```python
from build123d import *

# Parameters (mm, degrees)
SKETCH_1_R             = 12.5
EXTRUDE_1_DEPTH        = 298
SKETCH_2_R             = 10
EXTRUDE_2_DEPTH        = 56
EXTRUDE_START          = 56
SKETCH_3_R             = 10
EXTRUDE_3_DEPTH        = 56
SKETCH_4_R             = 7.5
EXTRUDE_4_DEPTH        = 5
EXTRUDE_START_2        = 5
SKETCH_5_R             = 7.5
EXTRUDE_5_DEPTH        = 5
HOLE_WIZARD_M8_1_D     = 6.8
HOLE_WIZARD_M8_1_DEPTH = 19.75
HOLE_WIZARD_M8_1_TIP   = 2.042926105
HOLE_WIZARD_M8_2_D     = 6.8
HOLE_WIZARD_M8_2_DEPTH = 19.75
HOLE_WIZARD_M8_2_TIP   = 2.042926105
CHAMFER_2_SIZE         = 0.5
CHAMFER_3_SIZE         = 0.5


with BuildPart() as part:
    # 草图1 → 凸台-拉伸1 (new body)
    with BuildSketch(Plane.XY):
        Circle(SKETCH_1_R)
    extrude(amount=EXTRUDE_1_DEPTH)

    # 草图2 → 凸台-拉伸2 (add)
    with BuildSketch(Plane(origin=(0, 0, 0), x_dir=(-1, 0, 0), z_dir=(0, 0, -1))):
        with Locations(Location((0, 0, 0), (0, 0, 180))):
            Circle(SKETCH_2_R)
    extrude(amount=EXTRUDE_2_DEPTH)

    # 草图3 → 凸台-拉伸3 (add)
    with BuildSketch(Plane.XY.offset(298).offset(EXTRUDE_START)):
        Circle(SKETCH_3_R)
    extrude(amount=-EXTRUDE_3_DEPTH)

    # 草图4 → 凸台-拉伸4 (add)
    with BuildSketch(Plane.XY.offset(354)):
        Circle(SKETCH_4_R)
    extrude(amount=EXTRUDE_4_DEPTH)

    # 草图5 → 凸台-拉伸5 (add)
    with BuildSketch(Plane(origin=(0, 0, -56), x_dir=(-1, 0, 0), z_dir=(0, 0, -1)).offset(EXTRUDE_START_2)):
        with Locations(Location((0, 0, 0), (0, 0, 180))):
            Circle(SKETCH_5_R)
    extrude(amount=-EXTRUDE_5_DEPTH)

    # M8 螺纹孔1
    with Locations(Plane(origin=(0, 0, -61), x_dir=(-1, 0, 0), z_dir=(0, 0, -1))):
        with Locations((0, 0)):
            Hole(HOLE_WIZARD_M8_1_D / 2, depth=HOLE_WIZARD_M8_1_DEPTH)
            with Locations((0, 0, -(HOLE_WIZARD_M8_1_DEPTH + HOLE_WIZARD_M8_1_TIP / 2))):  # 118° drill point
                Cone(0, HOLE_WIZARD_M8_1_D / 2, HOLE_WIZARD_M8_1_TIP, mode=Mode.SUBTRACT)

    # M8 螺纹孔2
    with Locations(Plane.XY.offset(359)):
        with Locations((0, 0)):
            Hole(HOLE_WIZARD_M8_2_D / 2, depth=HOLE_WIZARD_M8_2_DEPTH)
            with Locations((0, 0, -(HOLE_WIZARD_M8_2_DEPTH + HOLE_WIZARD_M8_2_TIP / 2))):  # 118° drill point
                Cone(0, HOLE_WIZARD_M8_2_D / 2, HOLE_WIZARD_M8_2_TIP, mode=Mode.SUBTRACT)

    # 倒角2
    chamfer_2_edges = [part.edges().sort_by_distance(p)[0] for p in [
        (-7.5, 0, 359),
    ]]
    chamfer(chamfer_2_edges, length=CHAMFER_2_SIZE)

    # 倒角3
    chamfer_3_edges = [part.edges().sort_by_distance(p)[0] for p in [
        (-7.5, 0, -61),
    ]]
    chamfer(chamfer_3_edges, length=CHAMFER_3_SIZE)


solid = part.part
```
Build history of the part. All positions in model axes, mm. A direction names the side the tool comes from. Round coordinates to 2 decimals unless told otherwise and drop trailing zeros. Order: outer loops, then holes, each group sorted by start corner. A loop starts at its lowest first (then second) coordinate and runs counter-clockwise, first axis right, second up. Notation, with made-up numbers: (10, -36.5) - (22, -36.5) arc R31 ccw to (22, -11.5) - close; hole circle Ø1 at (42.25, 16.25). An arc over 180 degrees is marked (long way). Use a Markdown table: item, result.
1) Saw through at A-A on z = -18. Write the cut outline in (x, y), and give its area (3 significant figures).
Recorded:
| item | result |
|---|---|
| outline | circle Ø20 at (0, 0) |
| area | 314 mm² |
2) Saw through at B-B on z = 136.5. Write the cut outline in (x, y), and give its area (3 significant figures).
Recorded:
| item | result |
|---|---|
| outline | circle Ø25 at (0, 0) |
| area | 491 mm² |
3) Flat gauge pins, fed straight in: pin 1 Ø8 at (x, z) = (6, 118) entering from +Y; pin 2 Ø5.5 at (x, y) = (0, 0) entering from +Z; pin 3 Ø3 at (x, z) = (-8.5, 86.5) entering from -Y. Where does each tip first touch, or does it go through?
Recorded:
| item | result |
|---|---|
| pin 1 | stops at y = 12.34 |
| pin 2 | stops at z = 338.86 |
| pin 3 | stops at y = -10.36 |
4) Tool access for faces 5 (the face through (4, -7, -56)), 6 (the face through (11.923, 3.755, 146.914)), 7 (the face through (-7.493, 0.33, 356.218)): list every direction of +Z, -Z, +X, -X, +Y, -Y with a clear straight run to the whole face (end or side of a thin tool).
Recorded:
| item | result |
|---|---|
| face 5 | -Z |
| face 6 | +Z, -Z |
| face 7 | +Z |
5) Wall check: L1, parallel to Y at x = 0, z = 343.75; L2, parallel to Z at x = 9.5, y = -6.75; L3, parallel to Y at x = -0.75, z = 337. Give the ranges that are in metal, low to high.
Recorded:
| item | result |
|---|---|
| L1 | y = -10 to -3.4, 3.4 to 10 |
| L2 | z = 0 to 298 |
| L3 | y = -9.97 to 9.97 |
6) Pull direction X, two halves, no side cores. Call faces 1 (the face through (4.032, -6.324, -58.282)), 2 (the face through (-0.1, 10.2, 298)), 3 (the face through (0.128, -0.576, -39.562)), 4 (the face through (-0.128, -0.576, 337.562)): pulls with the +X half, pulls with the -X half, needs draft (parallel to the pull), parting line crosses it, or undercut.
Recorded:
| item | result |
|---|---|
| face 1 | parting line crosses it |
| face 2 | needs draft |
| face 3 | undercut |
| face 4 | undercut |
